Input: part model. Units: mm. Frame: model coordinates. A direction names the side the tool comes from. Give positions to 0.01 mm unless a question says otherwise; leave off trailing zeros. Loops run counter-clockwise (first coordinate to the right, second up) from the corner with the lowest first, then second, coordinate; pieces in that order, holes last.
from build123d import *

# Parameters (mm, degrees)
EXTRUDE_START   = 13
SKETCH_2_R      = 30
EXTRUDE_1_DEPTH = 13


with BuildPart() as part:
    # 草图1 → 旋转1 (revolve)
    with BuildSketch(Plane(origin=(0, 0, 0), x_dir=(0, 0, -1), z_dir=(1, 0, 0)), mode=Mode.PRIVATE) as revolve_1_sk:
        with BuildLine():
            Line((-67, 28), (-67, 20))
            Line((-67, 20), (13, 20))
            Line((13, 20), (13, 28))
            ThreePointArc((13, 28), (12.414213562, 29.414213562), (11, 30))
            Line((11, 30), (-65, 30))
            ThreePointArc((-65, 30), (-66.414213562, 29.414213562), (-67, 28))
        make_face()
    revolve(revolve_1_sk.sketch.rotate(Axis((0, 0, -13), (0, 0, 1)), 90), axis=Axis((0, 0, -13), (0, 0, 1)))

    # 草图2 → 凸台-拉伸1 (add)
    with BuildSketch(Plane.XY.offset(EXTRUDE_START)):
        with BuildLine():
            Line((-33, 34.856850116), (-33, -34.856850116))
            ThreePointArc((-33, -34.856850116), (0, -48), (33, -34.856850116))
            Line((33, -34.856850116), (33, 34.856850116))
            ThreePointArc((33, 34.856850116), (0, 48), (-33, 34.856850116))
        make_face()
        with Locations(Location((0, 0, 0), (0, 0, 180))):
            Circle(SKETCH_2_R, mode=Mode.SUBTRACT)
    extrude(amount=-EXTRUDE_1_DEPTH)

    # 草图3 → 切除-旋转1 (revolve, cut)
    with BuildSketch(Plane(origin=(-22.5, 0, 0), x_dir=(0, 0, -1), z_dir=(1, 0, 0)), mode=Mode.PRIVATE) as cut_revolve_1_sk:
        Polygon((-13, 32), (-13, 39), (-4.9, 39), (-4.9, 36.5), (0, 36.5), (0, 32), align=None)
    revolve(cut_revolve_1_sk.sketch.rotate(Axis((-22.5, 32, 0), (0, 0, 1)), 90), axis=Axis((-22.5, 32, 0), (0, 0, 1)), mode=Mode.SUBTRACT)

    # 草图4 → 切除-旋转2 (revolve, cut)
    with BuildSketch(Plane(origin=(-22.5, 0, 0), x_dir=(0, 0, -1), z_dir=(1, 0, 0)), mode=Mode.PRIVATE) as cut_revolve_2_sk:
        Polygon((0, -32), (0, -36.5), (-4.9, -36.5), (-4.9, -39), (-13, -39), (-13, -32), align=None)
    revolve(cut_revolve_2_sk.sketch.rotate(Axis((-22.5, -32, 13), (0, 0, -1)), 270), axis=Axis((-22.5, -32, 13), (0, 0, -1)), mode=Mode.SUBTRACT)

    # 草图5 → 切除-旋转3 (revolve, cut)
    with BuildSketch(Plane(origin=(22.5, 0, 0), x_dir=(0, 0, -1), z_dir=(1, 0, 0)), mode=Mode.PRIVATE) as cut_revolve_3_sk:
        Polygon((-13, 32), (-13, 39), (-4.9, 39), (-4.9, 36.5), (0, 36.5), (0, 32), align=None)
    revolve(cut_revolve_3_sk.sketch.rotate(Axis((22.5, 32, 0), (0, 0, 1)), 90), axis=Axis((22.5, 32, 0), (0, 0, 1)), mode=Mode.SUBTRACT)

    # 草图6 → 切除-旋转4 (revolve, cut)
    with BuildSketch(Plane(origin=(22.5, 0, 0), x_dir=(0, 0, -1), z_dir=(1, 0, 0)), mode=Mode.PRIVATE) as cut_revolve_4_sk:
        Polygon((0, -32), (0, -36.5), (-4.9, -36.5), (-4.9, -39), (-13, -39), (-13, -32), align=None)
    revolve(cut_revolve_4_sk.sketch.rotate(Axis((22.5, -32, 13), (0, 0, -1)), 270), axis=Axis((22.5, -32, 13), (0, 0, -1)), mode=Mode.SUBTRACT)


solid = part.part
(1) Cut plane A-A (z = 9.5). Return the cut outline in (x, y), and give its area (3 significant figures).
Values follow:
outline: (-33, -34.86) arc R48 ccw to (33, -34.86) - (33, 34.86) arc R48 ccw to (-33, 34.86) - close; hole circle Ø14 at (-22.5, -32); hole circle Ø14 at (-22.5, 32); hole circle Ø40 at (0, 0); hole circle Ø14 at (22.5, -32); hole circle Ø14 at (22.5, 32)
area: 3,920 mm2
(2) Ray query, probe 1 along X at (y, z) = (-32, 3.3); probe 2 along X at (y, z) = (-32, 10); probe 3 along Y at (x, z) = (22.5, 1.2). Return the intervals inside material, ascending.
Values follow:
probe 1: x = -33 to -27, -18 to 18, 27 to 33
probe 2: x = -33 to -29.5, -15.5 to 15.5, 29.5 to 33
probe 3: y = -42.4 to -36.5, -27.5 to 27.5, 36.5 to 42.4
(3) Pin query (flat end, axial travel): pin 1 Ø2 at (x, z) = (0.5, 12.5) entering from -Y; pin 2 Ø12.5 at (x, y) = (-22.5, -32) entering from -Z; pin 3 Ø15.5 at (x, y) = (-25.5, -32.5) entering from +Z. Return the tip coordinate at first contact, or that it passes through.
Values follow:
pin 1: stops at y = -48
pin 2: stops at z = 0
pin 3: stops at z = 13
(4) Cut plane D-D (y = 32). Return the cut outline in (x, z), and give its area (3 significant figures).
Values follow:
outline: (-33, 0) - (-27, 0) - (-27, 4.9) - (-29.5, 4.9) - (-29.5, 13) - (-33, 13) - close; (-18, 0) - (18, 0) - (18, 4.9) - (15.5, 4.9) - (15.5, 13) - (-15.5, 13) - (-15.5, 4.9) - (-18, 4.9) - close; (27, 0) - (33, 0) - (33, 13) - (29.5, 13) - (29.5, 4.9) - (27, 4.9) - close
area: 543 mm2
(5) Cut plane C-C (x = 0). Return the cut outline in (y, z), and give its area (3 significant figures).
Values follow:
outline: (-48, 0) - (-30, 0) - (-30, -11) arc R2 ccw to (-28, -13) - (-20, -13) - (-20, 67) - (-28, 67) arc R2 ccw to (-30, 65) - (-30, 13) - (-48, 13) - close; (20, -13) - (28, -13) arc R2 ccw to (30, -11) - (30, 0) - (48, 0) - (48, 13) - (30, 13) - (30, 65) arc R2 ccw to (28, 67) - (20, 67) - close
area: 2,060 mm2
(6) Reachability of faces 1 (the cylindrical face through (21.52, -27.61, 2.48)), 2 (the flat face through (-22, -21, 0)), 3 (the cylindrical face through (-16.945, 36.259, 8.893)) from +Z, -Z, +X, -X, +Y, -Y: full face, straight path, thin tool, end or side. Return the list, or none.
Values follow:
face 1: +Z, -Z
face 2: -Z
face 3: +Z
(7) Cut plane B-B (y = 0). Return the cut outline in (x, z), and give its area (3 significant figures).
Values follow:
outline: (-33, 0) - (-30, 0) - (-30, -11) arc R2 ccw to (-28, -13) - (-20, -13) - (-20, 67) - (-28, 67) arc R2 ccw to (-30, 65) - (-30, 13) - (-33, 13) - close; (20, -13) - (28, -13) arc R2 ccw to (30, -11) - (30, 0) - (33, 0) - (33, 13) - (30, 13) - (30, 65) arc R2 ccw to (28, 67) - (20, 67) - close
area: 1,670 mm2
